Verification items for this drawing (mm, ordinates from the low corner). Coordinates: 2 decimals unless noted, no trailing zeros. Write each loop counter-clockwise with the first axis right and the second up, starting at its lowest first coordinate (ties: lowest second). Pieces come first, ordered by that corner, then holes.
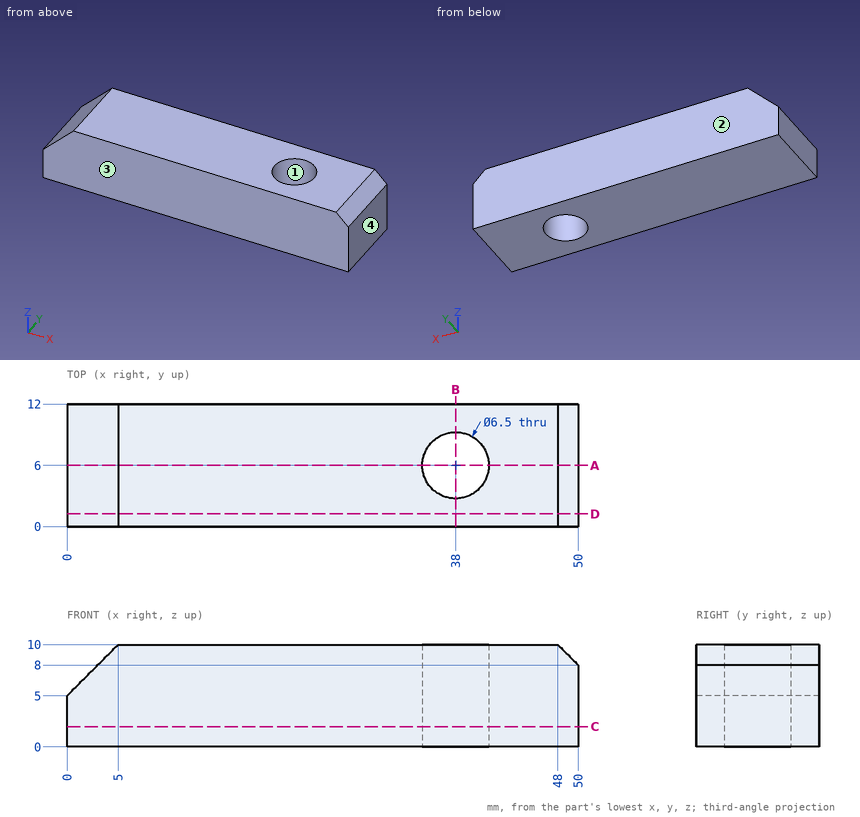
1. Sectioned sample at C-C, the plane z = 2. Record the boundary of the cut face in (x, y), and give its area (3 significant figures).
Computed values:
outline: (0, 0) - (50, 0) - (50, 12) - (0, 12) - close; hole circle Ø6.5 at (38, 6)
area: 567 mm2
2. Draft check along Y on the marked faces 1, 2, 3 and 4. Enter one of: released by +Y, released by -Y, zero draft, split by the parting line, or undercut.
Computed values:
face 1: undercut
face 2: released by +Y
face 3: released by -Y
face 4: zero draft
3. Sectioned sample at B-B, the plane x = 38. Record the boundary of the cut face in (y, z).
Computed values:
outline: (0, 0) - (2.75, 0) - (2.75, 10) - (0, 10) - close; (9.25, 0) - (12, 0) - (12, 10) - (9.25, 10) - close
4. Thickness scan on line 1 along Y through (x, z) = (38, 7.25); line 2 along X through (y, z) = (4, 1); line 3 along Y through (x, z) = (40, 6.5). Record the ranges inside material, lowest first.
Computed values:
line 1: y = 0 to 2.75, 9.25 to 12
line 2: x = 0 to 35.44, 40.56 to 50
line 3: y = 0 to 3.44, 8.56 to 12
5. Sectioned sample at D-D, the plane y = 1.25. Record the boundary of the cut face in (x, z).
Computed values:
outline: (0, 0) - (50, 0) - (50, 8) - (48, 10) - (5, 10) - (0, 5) - close
6. Sectioned sample at A-A, the plane y = 6. Record the boundary of the cut face in (x, z).
Computed values:
outline: (0, 0) - (34.75, 0) - (34.75, 10) - (5, 10) - (0, 5) - close; (41.25, 0) - (50, 0) - (50, 8) - (48, 10) - (41.25, 10) - close
